from build123d import *

# Parameters (mm, degrees)
BASE_BLOCK_SKETCH_W         = 56
BASE_BLOCK_SKETCH_H         = 35
BASE_BLOCK_DEPTH            = 110
BOTTOM_SLOT_SKETCH_W        = 20
BOTTOM_SLOT_SKETCH_H        = 15
BOTTOM_SLOT_DEPTH           = 110
SIDE_STEP_SKETCH_W          = 12
SIDE_STEP_SKETCH_H          = 15
SIDE_STEP_DEPTH             = 110
SIDE_LUG_1_DEPTH            = 16
SIDE_HOLE_1_SKETCH_R        = 7
SIDE_HOLE_1_DEPTH           = 16
SIDE_START                  = -16
SIDE_LUG_2_DEPTH            = 16
SIDE_HOLE_2_SKETCH_R        = 7
SIDE_HOLE_2_DEPTH           = 16
UPRIGHT_EAR_DEPTH           = 12
PIVOT_START                 = 8
PIVOT_BOSS_45_SKETCH_R      = 22.5
PIVOT_BOSS_45_DEPTH         = 8
PIVOT_BORE_20_SKETCH_R      = 10
PIVOT_BORE_20_DEPTH         = 20
COUNTERBORES_2X_24_SKETCH_R = 12
COUNTERBORES_2X_24_DEPTH    = 6
HOLES_2X_12_SKETCH_R        = 6
HOLES_2X_12_DEPTH           = 20


with BuildPart() as part:
    # Base Block Sketch → Base Block (new body)
    with BuildSketch(Plane.XY):
        with Locations((22, 17.5)):
            Rectangle(BASE_BLOCK_SKETCH_W, BASE_BLOCK_SKETCH_H)
    extrude(amount=BASE_BLOCK_DEPTH)

    # Bottom Slot Sketch → Bottom Slot (cut)
    with BuildSketch(Plane.XY.offset(110)):
        with Locations((20, 7.5)):
            Rectangle(BOTTOM_SLOT_SKETCH_W, BOTTOM_SLOT_SKETCH_H)
    extrude(amount=-BOTTOM_SLOT_DEPTH, mode=Mode.SUBTRACT)

    # Side Step Sketch → Side Step (add)
    with BuildSketch(Plane.XY.offset(110)):
        with Locations((0, 42.5)):
            Rectangle(SIDE_STEP_SKETCH_W, SIDE_STEP_SKETCH_H)
    extrude(amount=-SIDE_STEP_DEPTH)

    # Side Lug 1 Sketch → Side Lug 1 (add)
    with BuildSketch(Plane.XY.offset(110)):
        with BuildLine():
            Line((-45.151057186, 0), (-6, 0))
            Line((-6, 0), (-6, 50))
            Line((-6, 50), (-52.329877609, 26.455854883))
            ThreePointArc((-52.329877609, 26.455854883), (-59.498699864, 10.308671221), (-45.151057186, 0))
        make_face()
    extrude(amount=-SIDE_LUG_1_DEPTH)

    # Side Hole 1 Sketch → Side Hole 1 (cut)
    with BuildSketch(Plane.XY.offset(110)):
        with Locations((-45.987296801, 13.975002802)):
            Circle(SIDE_HOLE_1_SKETCH_R)
    extrude(amount=-SIDE_HOLE_1_DEPTH, mode=Mode.SUBTRACT)

    # Side Lug 2 Sketch → Side Lug 2 (add)
    with BuildSketch(Plane(origin=(0, 0, 0), x_dir=(-1, 0, 0), z_dir=(0, 0, -1)).offset(SIDE_START)):
        with BuildLine():
            Line((6, 50), (6, 0))
            Line((6, 0), (45.151057186, 0))
            ThreePointArc((45.151057186, 0), (59.498699864, 10.308671221), (52.329877609, 26.455854883))
            Line((52.329877609, 26.455854883), (6, 50))
        make_face()
    extrude(amount=SIDE_LUG_2_DEPTH)

    # Side Hole 2 Sketch → Side Hole 2 (cut)
    with BuildSketch(Plane(origin=(0, 0, 0), x_dir=(-1, 0, 0), z_dir=(0, 0, -1)).offset(SIDE_START)):
        with Locations(Location((45.987296801, 13.975002802, 0), (0, 0, 180))):
            Circle(SIDE_HOLE_2_SKETCH_R)
    extrude(amount=SIDE_HOLE_2_DEPTH, mode=Mode.SUBTRACT)

    # Upright Ear Sketch → Upright Ear (add)
    with BuildSketch(Plane.ZY.offset(6)):
        with BuildLine():
            Line((34.387072411, 92.019823514), (16, 50))
            Line((16, 50), (94, 50))
            Line((94, 50), (75.612927589, 92.019823514))
            ThreePointArc((75.612927589, 92.019823514), (55, 105.5), (34.387072411, 92.019823514))
        make_face()
    extrude(amount=-UPRIGHT_EAR_DEPTH)

    # Pivot Boss Ø45 Sketch → Pivot Boss Ø45 (add)
    with BuildSketch(Plane.ZY.offset(6).offset(PIVOT_START)):
        with Locations((55, 83)):
            Circle(PIVOT_BOSS_45_SKETCH_R)
    extrude(amount=-PIVOT_BOSS_45_DEPTH)

    # Pivot Bore Ø20 Sketch → Pivot Bore Ø20 (cut)
    with BuildSketch(Plane.ZY.offset(14)):
        with Locations((55, 83)):
            Circle(PIVOT_BORE_20_SKETCH_R)
    extrude(amount=-PIVOT_BORE_20_DEPTH, mode=Mode.SUBTRACT)

    # Counterbores 2xØ24 Sketch → Counterbores 2xØ24 (cut)
    with BuildSketch(Plane(origin=(0, 35, 0), x_dir=(1, 0, 0), z_dir=(0, 1, 0))):
        with Locations(Location((28, -90, 0), (0, 0, 270))):
            Circle(COUNTERBORES_2X_24_SKETCH_R)
        with Locations(Location((28, -55, 0), (0, 0, 270))):
            Circle(COUNTERBORES_2X_24_SKETCH_R)
    extrude(amount=-COUNTERBORES_2X_24_DEPTH, mode=Mode.SUBTRACT)

    # Holes 2xØ12 Sketch → Holes 2xØ12 (cut)
    with BuildSketch(Plane(origin=(0, 29, 0), x_dir=(1, 0, 0), z_dir=(0, 1, 0))):
        with Locations(Location((28, -55, 0), (0, 0, 270))):
            Circle(HOLES_2X_12_SKETCH_R)
        with Locations(Location((28, -90, 0), (0, 0, 270))):
            Circle(HOLES_2X_12_SKETCH_R)
    extrude(amount=-HOLES_2X_12_DEPTH, mode=Mode.SUBTRACT)


solid = part.part
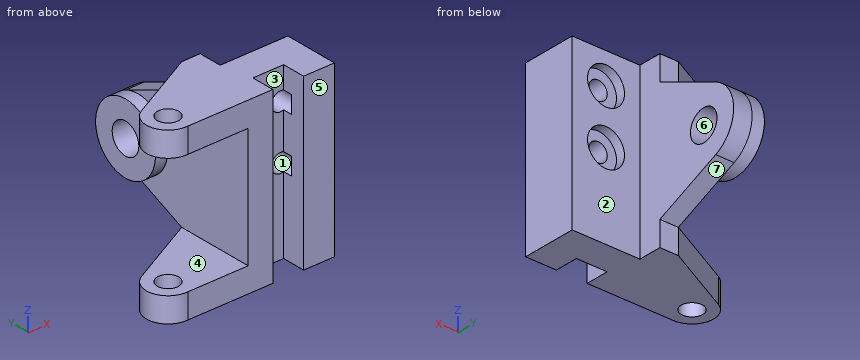
For this review, take the finished solid that the model builds, in its own axes (mm). Face numbers are marked on the shaded views. A direction names the side the tool comes from. Round coordinates to 2 decimals unless told otherwise and drop trailing zeros. Write each loop counter-clockwise with the first axis right and the second up, starting at its lowest first coordinate (ties: lowest second). Pieces come first, ordered by that corner, then holes. Notation, with made-up numbers: (54, 53) - (93, 53) arc R22 ccw to (93, 84) - close; hole circle Ø10 at (81.5, -7.75). An arc over 180 degrees is marked (long way). Use a Markdown table: item, result.
Q1. Machinability: for the marked faces 1, 2, 3 and 4, which of the approach directions +Z, -Z, +X, -X, +Y, -Y give a long, thin tool a straight path to every point of the face, cutting with its end or side? Answer none if there is none.
Derived:
| item | result |
|---|---|
| face 1 | +Y |
| face 2 | +Z, -Z, +X, +Y |
| face 3 | +Z, -Z, -Y |
| face 4 | -X, +Y, -Y |
Q2. We need section C-C (z = 55). Give the boundary of the cut face in (x, y).
Derived:
| item | result |
|---|---|
| outline | (-14, 60.5) - (-6, 60.5) - (-6, 0) - (10, 0) - (10, 15) - (22, 15) - (22, 29) - (16, 29) - (16, 35) - (6, 35) - (6, 73) - (-14, 73) - close; (-14, 93) - (6, 93) - (6, 105.5) - (-14, 105.5) - close; (30, 0) - (50, 0) - (50, 35) - (40, 35) - (40, 29) - (34, 29) - (34, 9) - (30, 9) - close |
Q3. We need section A-A (x = 28). Give the boundary of the cut face in (y, z).
Derived:
| item | result |
|---|---|
| outline | (15, 0) - (35, 0) - (35, 43) - (29, 43) - (29, 49) - (15, 49) - close; (15, 61) - (29, 61) - (29, 67) - (35, 67) - (35, 78) - (29, 78) - (29, 84) - (15, 84) - close; (15, 96) - (29, 96) - (29, 102) - (35, 102) - (35, 110) - (15, 110) - close |
Q4. The part is to be moulded in two halves that separate along Z. For the marked faces 5, 6 and 7, say which applies: pulls with the +Z half, pulls with the -Z half, needs draft (parallel to the pull), parting line crosses it, or undercut.
Derived:
| item | result |
|---|---|
| face 5 | needs draft |
| face 6 | undercut |
| face 7 | pulls with the -Z half |
Q5. We need section D-D (y = 31.5). Give the boundary of the cut face in (x, z).
Derived:
| item | result |
|---|---|
| outline | (-42.4, 0) - (50, 0) - (50, 110) - (-42.4, 110) - (-42.4, 94) - (-6, 94) - (-6, 16) - (-42.4, 16) - close; hole circle Ø24 at (28, 55); hole circle Ø24 at (28, 90) |
Q6. Wall thickness on line 1 along X through (y, z) = (14, 14.5); line 2 along Z through (x, y) = (-44.5, 26); line 3 along Z through (x, y) = (28, 20): over which ranges is each line inside the solid? List them lowest first.
Derived:
| item | result |
|---|---|
| line 1 | x = -59.99 to -52.99, -38.99 to 10, 30 to 50 |
| line 2 | z = 0 to 16, 94 to 110 |
| line 3 | z = 0 to 49, 61 to 84, 96 to 110 |
Q7. Clearance check with flat-ended pins moving along their axes: pin 1 (16.5 mm diameter, centred on y = 6.5, z = 45.5, fed in from -X); pin 2 (3 mm diameter, centred on x = 32.5, z = 87.5, fed in from +Y); pin 3 (1 mm diameter, centred on y = 72.5, z = 72, fed in from +X). State where each tip first meets the part, or that it passes through.
Derived:
| item | result |
|---|---|
| pin 1 | stops at x = -6 |
| pin 2 | stops at y = 29 |
| pin 3 | stops at x = 6 |
Q8. We need section B-B (x = 0.5). Give the boundary of the cut face in (y, z).
Derived:
| item | result |
|---|---|
| outline | (0, 0) - (50, 0) - (50, 16) - (92.02, 34.39) arc R22.5 ccw to (92.02, 75.61) - (50, 94) - (50, 110) - (0, 110) - close; hole circle Ø20 at (83, 55) |
